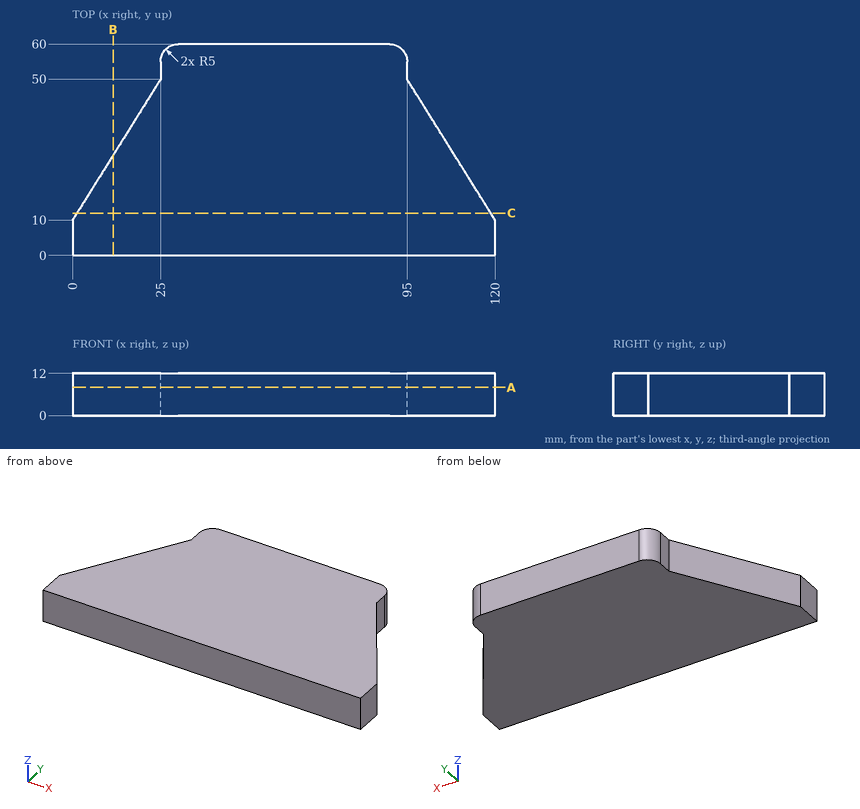
Study the drawing (mm; zero at the part's minimum x, y, z) and answer. Give positions to 0.01 mm unless a question says otherwise; leave off trailing zeros. Loops run counter-clockwise (first coordinate to the right, second up) from the corner with the lowest first, then second, coordinate; pieces in that order, holes last. Notation, with made-up numbers: M 5.5,49.5 L 32.5,49.5 A24 cw 32.5,81.5 Z; hole C 29,80 d11. An arc over 180 degrees is marked long. One line per item, written item: value. Start each with the question number.
1. Each of these flat-tipped pins is pushed along its axis until it touches: P1, Ø4, axis at x = 19.5, z = 4.5, coming from the -Y side; P2, Ø4, axis at y = 53.5, z = 8.5, coming from the +X side; P3, Ø4, axis at y = 32, z = 5, coming from the +X side; P4, Ø2, axis at y = 42, z = 2, coming from the +X side (3 decimals). Where does it stop, or does it pass through?
2. Find section B-B (x = 11.5). Give the vertices of the cut face in (y, z), and give its area (3 significant figures).
3. Find the intervals of material crossed by probe 1 along X at (y, z) = (55, 1.5); probe 2 along X at (y, z) = (36, 10.25); probe 3 along Y at (x, z) = (115.5, 3.5), in increasing order.
4. Find section A-A (z = 8). Give the vertices of the cut face in (x, y).
5. Find section C-C (y = 12). Give the vertices of the cut face in (x, z).
Reported:
1. P1: stops at y = 0
1. P2: stops at x = 95
1. P3: stops at x = 107.5
1. P4: stops at x = 100.625
2. outline: M 0,0 L 28.4,0 L 28.4,12 L 0,12 Z
2. area: 341 mm²
3. probe 1: x = 25 to 95
3. probe 2: x = 16.25 to 103.75
3. probe 3: y = 0 to 17.2
4. outline: M 0,0 L 120,0 L 120,10 L 95,50 L 95,55 A5 ccw 90,60 L 30,60 A5 ccw 25,55 L 25,50 L 0,10 Z
5. outline: M 1.25,0 L 118.75,0 L 118.75,12 L 1.25,12 Z
